Verification items for the finished model (mm, model axes). Give positions to 0.01 mm unless a question says otherwise; leave off trailing zeros. Write each loop counter-clockwise with the first axis right and the second up, starting at its lowest first coordinate (ties: lowest second). Pieces come first, ordered by that corner, then holes. Notation, with made-up numbers: (-20.5, 28) -> (34.5, 28) arc R15 cw to (34.5, 33) -> close; hole circle Ø1 at (69.25, -27.75). An arc over 180 degrees is marked (long way). Write item = value, one per line.
from build123d import *

# Parameters (mm, degrees)
EXTRUDE_1_DEPTH = 8


with BuildPart() as part:
    # 草图1 → 凸台-拉伸1 (new body)
    with BuildSketch(Plane(origin=(0, 0, 0), x_dir=(-1, 0, 0), z_dir=(0, 0, 1))):
        with BuildLine():
            Line((-176.477803528, -283.424824257), (-58.627916081, -240.213198859))
            ThreePointArc((-58.627916081, -240.213198859), (-44.360544026, -229.22495956), (-38.955555556, -212.046909383))
            Line((-38.955555556, -212.046909383), (-38.955555556, -193))
            Line((-38.955555556, -193), (-176.477803528, -193))
            Line((-176.477803528, -193), (-176.477803528, -283.424824257))
        make_face()
    extrude(amount=EXTRUDE_1_DEPTH)


solid = part.part
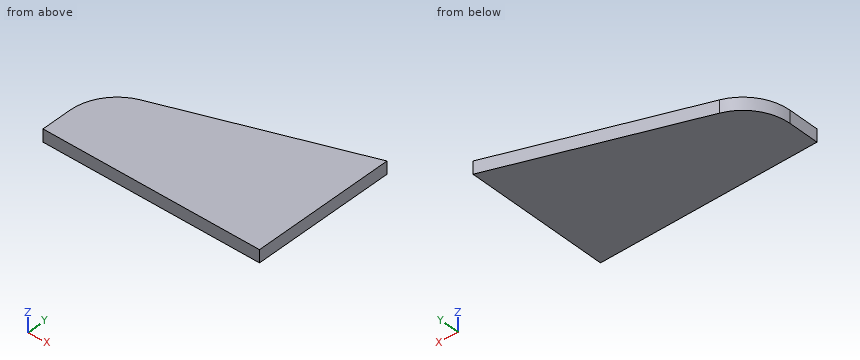
Item 1: Sectioned sample at A-A on z = 3.5. Record the cut outline in (x, y), then the cut area to 3 significant figures.
Response values:
outline = (38.96, 193) -> (176.48, 193) -> (176.48, 283.42) -> (58.63, 240.21) arc R30 ccw to (38.96, 212.05) -> close
area = 8,890 mm^2
Item 2: Sectioned sample at C-C on y = 266.5. Record the cut outline in (x, z), then the cut area to 3 significant figures.
Response values:
outline = (130.32, 0) -> (176.48, 0) -> (176.48, 8) -> (130.32, 8) -> close
area = 369 mm^2
Item 3: Go/stop test with flat-tipped pins: P1, Ø1.5, axis at x = 98, z = 1, coming from the +Y side; P2, Ø3, axis at x = 79, z = 2.5, coming from the +Y side. Record where each tip stops, or that it passes through.
Response values:
P1 = 254.92
P2 = 248.23
Item 4: Sectioned sample at B-B on x = 121. Record the cut outline in (y, z).
Response values:
outline = (193, 0) -> (263.08, 0) -> (263.08, 8) -> (193, 8) -> close
Item 5: Material ranges on line 1 (Y direction, x = 121, z = 4.5); line 2 (Y direction, x = 55, z = 6.5); line 3 (X direction, y = 238, z = 7.25), recorded low to high.
Response values:
line_1 = 193 to 263.08
line_2 = 193 to 238.6
line_3 = 53.91 to 176.48
